Source: three-view drawing plus pictorial views. Frame: mm from the lowest corner of the part. Round coordinates to 2 decimals unless told otherwise and drop trailing zeros. Loops run counter-clockwise (first coordinate to the right, second up) from the corner with the lowest first, then second, coordinate; pieces in that order, holes last. Notation, with made-up numbers: (58, -38) -> (109, -38) arc R25 cw to (109, -17) -> close; hole circle Ø4 at (16.25, 12.5). An arc over 180 degrees is marked (long way). Return JSON: item names as keys, results as strings. Group by question number.
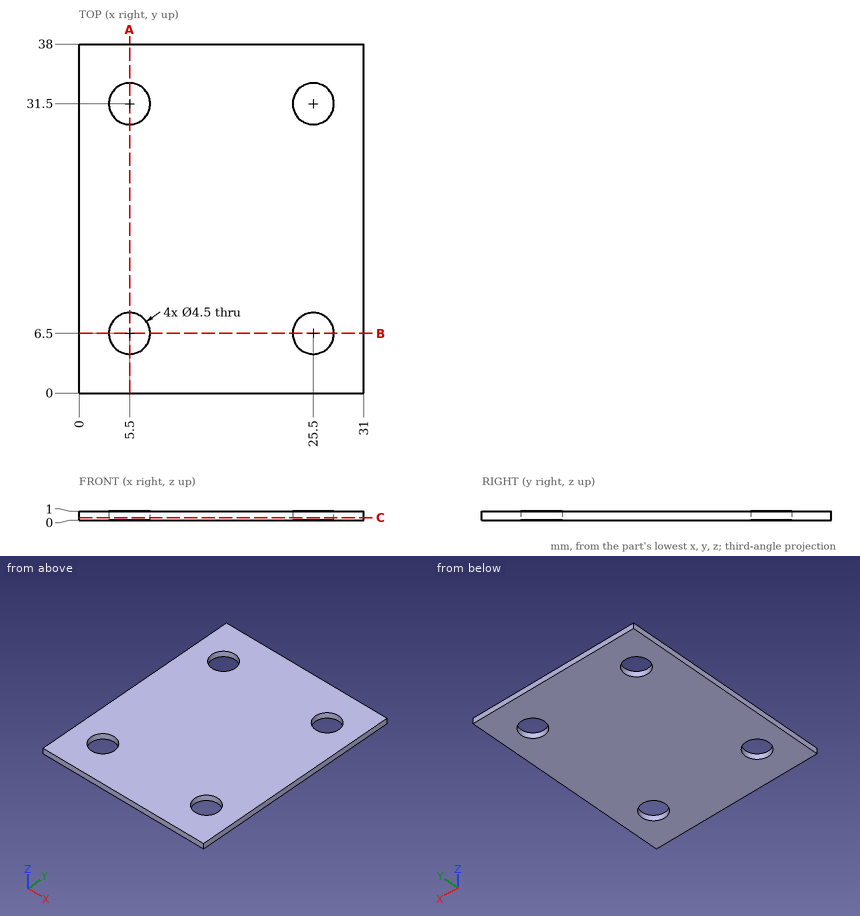
(1) Cut plane A-A (x = 5.5). Return loops of the section in (y, z).
(2) Pin query (flat end, axial travel): pin 1 (7 mm diameter, centred on x = 5.5, y = 6.5, fed in from +Z). Return the tip coordinate at first contact, or that it passes through.
(3) Cut plane B-B (y = 6.5). Return loops of the section in (x, z).
(4) Cut plane C-C (z = 0.3). Return loops of the section in (x, y).
(5) Ray query, line 1 (Y direction, x = 5.5, z = 0.5); line 2 (Y direction, x = 4.5, z = 0.85); line 3 (X direction, y = 32.5, z = 0.7). Return the intervals inside material, ascending.
Answers follow:
{
 "1": {"outline": "(0, 0) -> (4.25, 0) -> (4.25, 1) -> (0, 1) -> close; (8.75, 0) -> (29.25, 0) -> (29.25, 1) -> (8.75, 1) -> close; (33.75, 0) -> (38, 0) -> (38, 1) -> (33.75, 1) -> close"},
 "2": {"pin 1": "z = 1"},
 "3": {"outline": "(0, 0) -> (3.25, 0) -> (3.25, 1) -> (0, 1) -> close; (7.75, 0) -> (23.25, 0) -> (23.25, 1) -> (7.75, 1) -> close; (27.75, 0) -> (31, 0) -> (31, 1) -> (27.75, 1) -> close"},
 "4": {"outline": "(0, 0) -> (31, 0) -> (31, 38) -> (0, 38) -> close; hole circle Ø4.5 at (5.5, 6.5); hole circle Ø4.5 at (5.5, 31.5); hole circle Ø4.5 at (25.5, 6.5); hole circle Ø4.5 at (25.5, 31.5)"},
 "5": {"line 1": "0 to 4.25, 8.75 to 29.25, 33.75 to 38", "line 2": "0 to 4.48, 8.52 to 29.48, 33.52 to 38", "line 3": "0 to 3.48, 7.52 to 23.48, 27.52 to 31"}
}
